Build history of the part. All positions in model axes, mm. Face numbers are marked on the shaded views. A direction names the side the tool comes from. Give positions to 0.01 mm unless a question says otherwise; leave off trailing zeros. Loops run counter-clockwise (first coordinate to the right, second up) from the corner with the lowest first, then second, coordinate; pieces in that order, holes last. Notation, with made-up numbers: M 22,26 L 35,26 A20 cw 35,57 Z; hole C -19.5,1 d9. An arc over 180 degrees is marked long. Put each result on its own line as item: value.
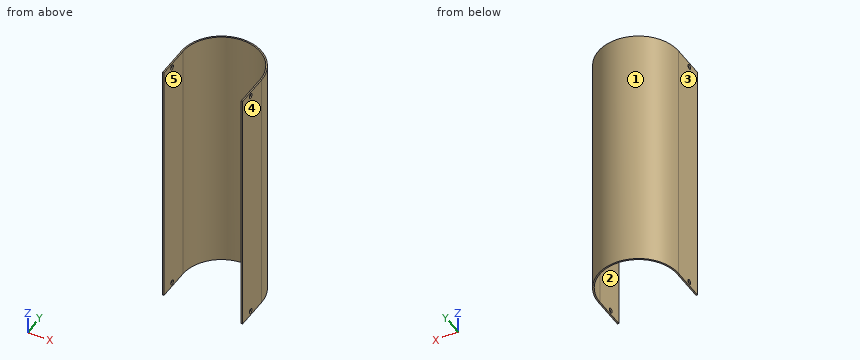
```python
from build123d import *

# Parameters (mm, degrees)
EXTRUDE_1_DEPTH     = 265
SKETCH_2_R          = 2.5
CUT_EXTRUDE_1_DEPTH = 289.461435897


with BuildPart() as part:
    # 草图1 → 凸台-拉伸1 (new body)
    with BuildSketch(Plane.XY):
        with BuildLine():
            Line((-20.582221357, 0), (-19.082221357, 0))
            Line((-19.082221357, 0), (-19.082221357, 35))
            ThreePointArc((-19.082221357, 35), (21.417778643, 75.5), (61.917778643, 35))
            Line((61.917778643, 35), (61.917778643, 0))
            Line((61.917778643, 0), (63.417778643, 0))
            Line((63.417778643, 0), (63.417778643, 35))
            ThreePointArc((63.417778643, 35), (21.417778643, 77), (-20.582221357, 35))
            Line((-20.582221357, 35), (-20.582221357, 0))
        make_face()
    extrude(amount=EXTRUDE_1_DEPTH)

    # 草图2 → 切除-拉伸1 (cut, through all)
    with BuildSketch(Plane(origin=(63.417778643, 0, 0), x_dir=(0, 0, -1), z_dir=(1, 0, 0))):
        with Locations(Location((-260.5, 15, 0), (0, 0, 90))):
            Circle(SKETCH_2_R)
        with Locations(Location((-4.5, 15, 0), (0, 0, 90))):
            Circle(SKETCH_2_R)
    extrude(amount=-CUT_EXTRUDE_1_DEPTH, mode=Mode.SUBTRACT)


solid = part.part
```
Q1. Slice it at C-C (y = 32). List the corners of the cut face in (x, z).
Here are the results:
outline: M -20.58,0 L -19.08,0 L -19.08,265 L -20.58,265 Z; M 61.92,0 L 63.42,0 L 63.42,265 L 61.92,265 Z
Q2. Slice it at A-A (y = 15). List the corners of the cut face in (x, z).
Here are the results:
outline: M -20.58,0 L -19.08,0 L -19.08,2 L -20.58,2 Z; M -20.58,7 L -19.08,7 L -19.08,258 L -20.58,258 Z; M -20.58,263 L -19.08,263 L -19.08,265 L -20.58,265 Z; M 61.92,0 L 63.42,0 L 63.42,2 L 61.92,2 Z; M 61.92,7 L 63.42,7 L 63.42,258 L 61.92,258 Z; M 61.92,263 L 63.42,263 L 63.42,265 L 61.92,265 Z
Q3. Drop flat-ended pins along their axis: pin 1 Ø3 at (x, z) = (-12, 206) entering from +Y; pin 2 Ø1 at (y, z) = (64.5, 200.5) entering from -X; pin 3 Ø2 at (x, z) = (34.5, 117) entering from -Y; pin 4 Ø4.5 at (y, z) = (15, 4.5) entering from -X. Give the stop position or say it passes through.
Here are the results:
pin 1: y = 62.3
pin 2: x = -8.96
pin 3: y = 72.97
pin 4: through
Q4. Mould opens along X. For the marked faces 3, 4 and 5 say: pulls with the +X half, pulls with the -X half, needs draft (parallel to the pull), parting line crosses it, or undercut.
Here are the results:
face 3: pulls with the -X half
face 4: pulls with the +X half
face 5: undercut
Q5. Tool access for the marked faces 1 and 2: list every direction of +Z, -Z, +X, -X, +Y, -Y with a clear straight run to the whole face (end or side of a thin tool).
Here are the results:
face 1: +Z, -Z, +Y
face 2: +Z, -Z, -Y
Q6. Probe line 1 (Z direction, x = 62.4, y = 15); line 2 (X direction, y = 4.5, z = 82); line 3 (X direction, y = 65.5, z = 128.5). List the from-to ranges inside material, lowest first. Write a range as from..to.
Here are the results:
line 1: 0..2, 7..258, 263..265
line 2: -20.58..-19.08, 61.92..63.42
line 3: -7.46..-5.23, 48.06..50.29
Q7. Slice it at D-D (z = 209). List the corners of the cut face in (x, y), and give its area (3 significant figures).
Here are the results:
outline: M -20.58,0 L -19.08,0 L -19.08,35 A40.5 cw 61.92,35 L 61.92,0 L 63.42,0 L 63.42,35 A42 ccw -20.58,35 Z
area: 299 mm²
Q8. Slice it at B-B (z = 260.5). List the corners of the cut face in (x, y), and give its area (3 significant figures).
Here are the results:
outline: M -20.58,0 L -19.08,0 L -19.08,12.5 L -20.58,12.5 Z; M -20.58,17.5 L -19.08,17.5 L -19.08,35 A40.5 cw 61.92,35 L 61.92,17.5 L 63.42,17.5 L 63.42,35 A42 ccw -20.58,35 Z; M 61.92,0 L 63.42,0 L 63.42,12.5 L 61.92,12.5 Z
area: 284 mm²
